from build123d import *

# Parameters (mm, degrees)
SKETCH2_R           = 17.5
CUT_EXTRUDE1_DEPTH  = 15
SKETCH3_R           = 9
BOSS_EXTRUDE1_DEPTH = 1
SKETCH4_R           = 7
CUT_EXTRUDE2_DEPTH  = 37.715119501
SKETCH5_R           = 2
CUT_EXTRUDE3_DEPTH  = 4
CIRPATTERN1_COUNT   = 8
CIRPATTERN2_COUNT   = 4
CHAMFER1_SIZE       = 0.5


with BuildPart() as part:
    # Sketch1 → Revolve1 (revolve)
    with BuildSketch(Plane(origin=(0, 0, 0), x_dir=(0, 0, -1), z_dir=(1, 0, 0))):
        Polygon((0, 0), (-18, 0), (-18, 2), (-20, 2), (-24, 9), (-24, 23), (0, 23), align=None)
    revolve(axis=Axis((0, 23, 0), (0, -1, 0)))

    # Sketch2 → Cut-Extrude1 (cut)
    with BuildSketch(Plane(origin=(0, 23, 0), x_dir=(1, 0, 0), z_dir=(0, 1, 0))):
        with Locations(Location((0, 0, 0), (0, 0, 270))):
            Circle(SKETCH2_R)
    extrude(amount=-CUT_EXTRUDE1_DEPTH, mode=Mode.SUBTRACT)

    # Sketch3 → Boss-Extrude1 (add)
    with BuildSketch(Plane(origin=(0, 8, 0), x_dir=(1, 0, 0), z_dir=(0, 1, 0))):
        with Locations(Location((0, 0, 0), (0, 0, 270))):
            Circle(SKETCH3_R)
    extrude(amount=BOSS_EXTRUDE1_DEPTH)

    # Sketch4 → Cut-Extrude2 (cut, through all)
    with BuildSketch(Plane(origin=(0, 9, 0), x_dir=(1, 0, 0), z_dir=(0, 1, 0))):
        with Locations(Location((0, 0, 0), (0, 0, 270))):
            Circle(SKETCH4_R)
    extrude(amount=-CUT_EXTRUDE2_DEPTH, mode=Mode.SUBTRACT)

    # Sketch5 → Cut-Extrude3 (cut)
    with BuildSketch(Plane.XZ):
        with Locations(Location((0, 14, 0), (0, 0, 270))):
            Circle(SKETCH5_R)
    extrude(amount=-CUT_EXTRUDE3_DEPTH, mode=Mode.SUBTRACT)

    # Sketch6 → Cut-Revolve1 (revolve, cut)
    with BuildSketch(Plane.XY):
        with BuildLine():
            Line((-16, 0), (-14, 0))
            Line((-14, 0), (-14, 1))
            ThreePointArc((-14, 1), (-15.104156256, 0.708312513), (-16, 0))
        make_face()
    cut_revolve1 = revolve(axis=Axis((-14, 0, 0), (0, 1, 0)), mode=Mode.SUBTRACT)

    # CirPattern1: Cut-Revolve1 ×8 about axis, 2 skipped
    cirpattern1_axis = Axis((0, 0, 0), (0, 1, 0))
    add([cut_revolve1.rotate(cirpattern1_axis, i * 360 / CIRPATTERN1_COUNT) for i in range(1, CIRPATTERN1_COUNT) if i not in (2, 6)], mode=Mode.SUBTRACT)

    # Sketch8 → M4 Tapped Hole1 (revolve, cut)
    with BuildSketch(Plane(origin=(0, 23, -20.75), x_dir=(0, 0, 1), z_dir=(1, 0, 0))):
        Polygon((0, 0), (0, 8.991420021), (1.65, 8), (1.65, 0.375), (2.025, 0), align=None)
    m4_tapped_hole1 = revolve(axis=Axis((0, 29.35, -20.75), (0, -1, 0)), mode=Mode.SUBTRACT)

    # CirPattern2: M4 Tapped Hole1 ×4 about axis
    cirpattern2_axis = Axis((0, 0, 0), (0, 1, 0))
    for i in range(1, CIRPATTERN2_COUNT):
        add(m4_tapped_hole1.rotate(cirpattern2_axis, i * 360 / CIRPATTERN2_COUNT), mode=Mode.SUBTRACT)

    # Chamfer1
    chamfer1_edges = [part.edges().sort_by_distance(p)[0] for p in [
        (0, 0, -7),
    ]]
    chamfer(chamfer1_edges, length=CHAMFER1_SIZE)


solid = part.part
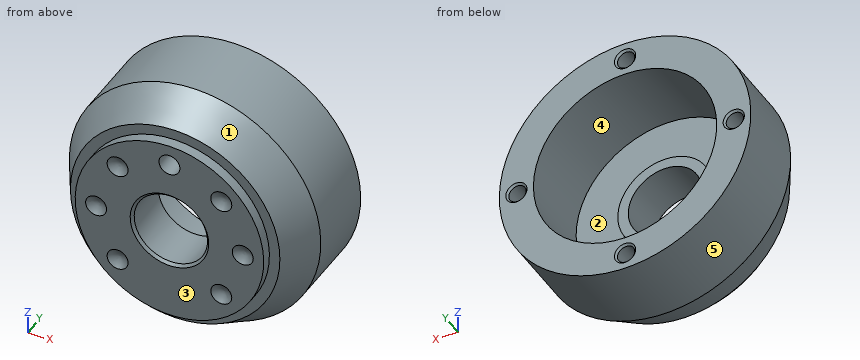
Part model, mm, in its own coordinate system. Face numbers are marked on the shaded views. A direction names the side the tool comes from. Round coordinates to 2 decimals unless told otherwise and drop trailing zeros. Write each loop counter-clockwise with the first axis right and the second up, starting at its lowest first coordinate (ties: lowest second). Pieces come first, ordered by that corner, then holes. Notation, with made-up numbers: M 29,-1.75 L 57,-1.75 A17 cw 57,3.25 Z; hole C 73.25,53.25 d2. An arc over 180 degrees is marked long. Return JSON: item names as keys, results as strings. Group by question number.
(1) Pin check, flat tips, straight feed: pin 1 Ø5 at (x, z) = (3, 7.5) entering from -Y; pin 2 Ø2 at (x, z) = (0, 20.75) entering from +Y; pin 3 Ø8 at (y, z) = (8, 18) entering from +X; pin 4 Ø5 at (x, y) = (14, 18.5) entering from -Z. Stop position of each tip, or through.
(2) Drill centre lines: probe 1 along Z at (x, y) = (0.5, 16.75); probe 2 along Y at (x, z) = (-0.5, 13.5); probe 3 along Z at (x, y) = (-20.75, 20). Where is each one in solid material? Low to high.
(3) Which spindle directions (+Z, -Z, +X, -X, +Y, -Y) get a long thin tool onto all of the face, cutting with end or side? Do the marked faces 4 and 5. Say none if no direction does.
(4) Two-plate mould, pull along X, no slides. Class the marked faces 1, 2 and 3: +X half, -X half, draft (parallel to the pull), parting line (faces both ways), or undercut.
(5) Saw through at A-A on y = 10.75. Write the cut outline in (x, z), then the cut area to 3 significant figures.
Returned:
{
 "1": {"pin 1": "y = 0", "pin 2": "y = 14.61", "pin 3": "x = 19.4", "pin 4": "z = -21.07"},
 "2": {"probe 1": "-23.99 to -22.32, -19.18 to -17.49, 17.49 to 19.18, 22.32 to 23.99", "probe 2": "4 to 8", "probe 3": "-12.06 to -1.65, 1.65 to 12.06"},
 "3": {"face 4": "+Y", "face 5": "+Y, -Y"},
 "4": {"face 1": "parting line", "face 2": "undercut", "face 3": "draft"},
 "5": {"outline": "C 0,0 d48; hole C 0,0 d35", "area": "847 mm²"}
}
